from build123d import *


with BuildPart() as part:
    # Piston Profile Sketch → Piston Body Revolve (revolve)
    with BuildSketch(Plane.XY, mode=Mode.PRIVATE) as piston_body_revolve_sk:
        with BuildLine():
            Line((0, 0), (37, 0))
            Line((37, 0), (42, 0))
            Line((42, 0), (42, 5))
            Line((42, 5), (38, 5))
            Line((38, 5), (38, 7))
            Line((38, 7), (42, 7))
            Line((42, 7), (42, 9))
            Line((42, 9), (38, 9))
            Line((38, 9), (38, 50))
            Line((38, 50), (42, 50))
            Line((42, 50), (42, 52))
            Line((42, 52), (38, 52))
            Line((38, 52), (38, 55))
            Line((38, 55), (42, 55))
            Line((42, 55), (42, 57))
            Line((42, 57), (38, 57))
            Line((38, 57), (38, 60))
            Line((38, 60), (42, 60))
            Line((42, 60), (42, 62))
            Line((42, 62), (38, 62))
            Line((38, 62), (38, 65))
            Line((38, 65), (42, 65))
            Line((42, 65), (42, 67.182193635))
            Line((42, 67.182193635), (38, 67.182193635))
            ThreePointArc((38, 67.182193635), (19, 69.801945586), (0, 67.182193635))
            Line((0, 67.182193635), (0, 0))
        make_face()
    revolve(piston_body_revolve_sk.sketch.rotate(Axis((0, 0, 0), (0, 1, 0)), 90), axis=Axis((0, 0, 0), (0, 1, 0)))


solid = part.part
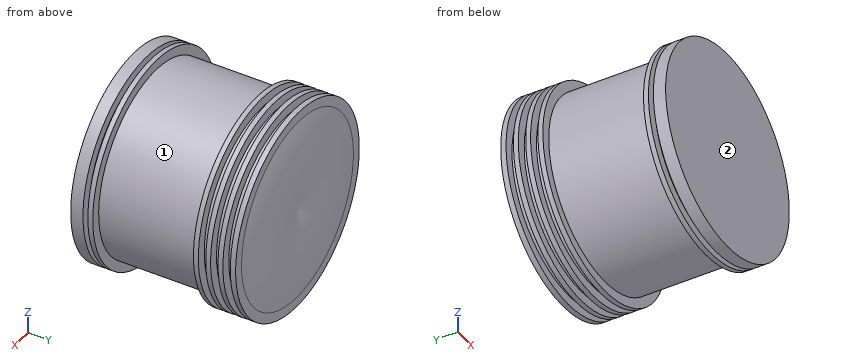
Design review of the part built by this model. Coordinates are the model's own, in mm. Face numbers are marked on the shaded views. A direction names the side the tool comes from. Give positions to 0.01 mm unless a question says otherwise; leave off trailing zeros. Order: outer loops, then holes, each group sorted by start corner. A loop starts at its lowest first (then second) coordinate and runs counter-clockwise, first axis right, second up. Notation, with made-up numbers: (47, 55.5) - (74, 55.5) arc R26 ccw to (74, 93.5) - close; hole circle Ø8 at (-4.75, -21). An arc over 180 degrees is marked (long way). Write item = value, one per line. Start each with the question number.
Q1. Clearance check with flat-ended pins moving along their axes: pin 1 Ø6 at (y, z) = (24.5, 32) entering from +X; pin 2 Ø2 at (x, y) = (2.5, 14) entering from +Z; pin 3 Ø1 at (x, y) = (-9.5, 25.5) entering from -Z; pin 4 Ø25 at (x, z) = (-12, 0.5) entering from -Y. State where each tip first meets the part, or that it passes through.
Q2. To check wall thickness, follow L1, parallel to Y at x = 17, z = -36.5; L2, parallel to X at y = 61.5, z = 0; L3, parallel to Y at x = -10, z = -14. State the ranges of each line that lie inside material, in increasing order. Write a range as from..to.
Q3. Tool access review of the marked faces 1 and 2: name each direction out of +Z, -Z, +X, -X, +Y, -Y from which nothing blocks a thin tool from reaching the whole face with its end or side.
Q4. We need section A-A on y = 18. State the section outline as (x, z) points.
Working result:
q1.pin_1 = 24.56
q1.pin_2 = 37.97
q1.pin_3 = -36.92
q1.pin_4 = 0
q2.L1 = 0..5, 7..9, 50..52, 55..57, 60..62, 65..67.18
q2.L2 = -42..42
q2.L3 = 0..69.78
q3.face_1 = none
q3.face_2 = +Z, -Z, +X, -X, -Y
q4.outline = circle Ø76 at (0, 0)
